```python
from build123d import *

# Parameters (mm, degrees)
SKETCH1_W           = 22
SKETCH1_H           = 22
BOSS_EXTRUDE1_DEPTH = 226.5
SKETCH2_R           = 6
CUT_EXTRUDE1_DEPTH  = 228.831626426
CHAMFER1_SIZE       = 5
CHAMFER2_SIZE       = 12


with BuildPart() as part:
    # Sketch1 → Boss-Extrude1 (new, symmetric)
    with BuildSketch(Plane.XY):
        Rectangle(SKETCH1_W, SKETCH1_H)
    extrude(amount=BOSS_EXTRUDE1_DEPTH, both=True)

    # Sketch2 → Cut-Extrude1 (cut, through all)
    with BuildSketch(Plane(origin=(0, 11, 0), x_dir=(1, 0, 0), z_dir=(0, 1, 0))):
        with Locations(Location((0, -196.5, 0), (0, 0, 270))):
            Circle(SKETCH2_R)
        with Locations(Location((0, -112.5, 0), (0, 0, 270))):
            Circle(SKETCH2_R)
        with Locations(Location((0, 83.5, 0), (0, 0, 270))):
            Circle(SKETCH2_R)
        with Locations(Location((0, 167.5, 0), (0, 0, 270))):
            Circle(SKETCH2_R)
    extrude(amount=-CUT_EXTRUDE1_DEPTH, mode=Mode.SUBTRACT)

    # Chamfer1
    chamfer1_edges = [part.edges().sort_by_distance(p)[0] for p in [
        (0, -11, 226.5),
    ]]
    chamfer(chamfer1_edges, length=CHAMFER1_SIZE)

    # Chamfer2
    chamfer2_edges = [part.edges().sort_by_distance(p)[0] for p in [
        (0, 11, -226.5),
    ]]
    chamfer(chamfer2_edges, length=CHAMFER2_SIZE)


solid = part.part
```
Read the model definition and answer for the solid it produces. Units are mm, in the model's axes. Coordinates: 2 decimals unless noted, no trailing zeros. Write each loop counter-clockwise with the first axis right and the second up, starting at its lowest first coordinate (ties: lowest second). Pieces come first, ordered by that corner, then holes. Notation, with made-up numbers: (25.5, 4.25) -> (64.5, 4.25) arc R22 cw to (64.5, 19.25) -> close; hole circle Ø11 at (42.5, 81). An arc over 180 degrees is marked (long way). Return JSON: item names as keys, results as strings.
1. A cutting plane is placed at C-C (y = 4.75). Determine the outline of the cut face in (x, z), and give its area (3 significant figures).
Found:
{"outline": "(-11, -220.75) -> (11, -220.75) -> (11, 226.5) -> (-11, 226.5) -> close; hole circle Ø12 at (0, -167.5); hole circle Ø12 at (0, -83.5); hole circle Ø12 at (0, 112.5); hole circle Ø12 at (0, 196.5)", "area": "9,390 mm2"}
2. Determine the mould class of faces 1 (the face through (0.264, 0.154, -89.494)), 2 (the face through (-0.2, 5.1, -220.4)), 3 (the face through (11, 0, 3)), 4 (the face through (-11, 0, 3)) for opening direction X: pulls with the +X half, pulls with the -X half, needs draft (parallel to the pull), parting line crosses it, or undercut.
Found:
{"face 1": "undercut", "face 2": "needs draft", "face 3": "pulls with the +X half", "face 4": "pulls with the -X half"}
3. Find the intervals of material crossed by line 1 along Z through (x, y) = (-3, 6.25); line 2 along X through (y, z) = (1.75, -83.5); line 3 along Z through (x, y) = (3.25, -4.75), in increasing order. Write a range as from..to.
Found:
{"line 1": "-219.25..-172.7, -162.3..-88.7, -78.3..107.3, 117.7..191.3, 201.7..226.5", "line 2": "-11..-6, 6..11", "line 3": "-226.5..-172.54, -162.46..-88.54, -78.46..107.46, 117.54..191.46, 201.54..226.5"}
4. A cutting plane is placed at B-B (z = 196.5). Determine the outline of the cut face in (x, y).
Found:
{"outline": "(-11, -11) -> (-6, -11) -> (-6, 11) -> (-11, 11) -> close; (6, -11) -> (11, -11) -> (11, 11) -> (6, 11) -> close"}
5. A cutting plane is placed at A-A (x = 0). Determine the outline of the cut face in (y, z).
Found:
{"outline": "(-11, -226.5) -> (-1, -226.5) -> (11, -214.5) -> (11, -173.5) -> (-11, -173.5) -> close; (-11, -161.5) -> (11, -161.5) -> (11, -89.5) -> (-11, -89.5) -> close; (-11, -77.5) -> (11, -77.5) -> (11, 106.5) -> (-11, 106.5) -> close; (-11, 118.5) -> (11, 118.5) -> (11, 190.5) -> (-11, 190.5) -> close; (-11, 202.5) -> (11, 202.5) -> (11, 226.5) -> (-6, 226.5) -> (-11, 221.5) -> close"}
